```python
from build123d import *

# Parameters (mm, degrees)
SKETCH_1_W                   = 30
SKETCH_1_H                   = 40
EXTRUDE_1_DEPTH              = 9
SKETCH_2_W                   = 30
SKETCH_2_H                   = 12
EXTRUDE_2_DEPTH              = 10
HOLE_WIZARD_M4_1_D           = 4.5
HOLE_WIZARD_M4_1_CBORE_D     = 8
HOLE_WIZARD_M4_1_CBORE_DEPTH = 4.4
CHAMFER_1_SIZE               = 1
CUT_EXTRUDE_1_DEPTH          = 32.400636936


with BuildPart() as part:
    # 草图1 → 凸台-拉伸1 (new body)
    with BuildSketch(Plane(origin=(0, 0, 0), x_dir=(1, 0, 0), z_dir=(0, 1, 0))):
        Rectangle(SKETCH_1_W, SKETCH_1_H)
    extrude(amount=EXTRUDE_1_DEPTH)

    # 草图2 → 凸台-拉伸2 (add)
    with BuildSketch(Plane(origin=(0, 9, 0), x_dir=(1, 0, 0), z_dir=(0, 1, 0))):
        with Locations((0, 14)):
            Rectangle(SKETCH_2_W, SKETCH_2_H)
    extrude(amount=EXTRUDE_2_DEPTH)

    # M4 六角凹头螺钉的柱形沉头孔1 (through all)
    with Locations(Plane(origin=(0, 0, 0), x_dir=(-1, 0, 0), z_dir=(0, -1, 0))):
        with Locations((-10, 15), (10, 15)):
            CounterBoreHole(HOLE_WIZARD_M4_1_D / 2, HOLE_WIZARD_M4_1_CBORE_D / 2, HOLE_WIZARD_M4_1_CBORE_DEPTH)

    # 倒角1
    chamfer_1_edges = [part.edges().sort_by_distance(p)[0] for p in [
        (-15, 14, -8),
        (15, 14, -8),
        (-15, 9.5, -20),
        (15, 9.5, -20),
        (15, 4.5, 20),
        (-15, 4.5, 20),
    ]]
    chamfer(chamfer_1_edges, length=CHAMFER_1_SIZE)

    # 草图5 → 切除-拉伸1 (cut, through all)
    with BuildSketch(Plane.XZ):
        with BuildLine():
            Line((2.5, 20), (2.5, 10))
            ThreePointArc((2.5, 10), (0, 7.5), (-2.5, 10))
            Line((-2.5, 10), (-2.5, 20))
            ThreePointArc((-2.5, 20), (0, 22.5), (2.5, 20))
        make_face()
    extrude(amount=-CUT_EXTRUDE_1_DEPTH, mode=Mode.SUBTRACT)


solid = part.part
```
Geometry check sheet. Reference: the model listing, model coordinates, mm. A direction names the side the tool comes from. Round coordinates to 2 decimals unless told otherwise and drop trailing zeros. Loops run counter-clockwise (first coordinate to the right, second up) from the corner with the lowest first, then second, coordinate; pieces in that order, holes last. Notation, with made-up numbers: (52, 31.25) - (72, 31.25) arc R25 cw to (72, 46.25) - close; hole circle Ø10 at (77.25, 20). An arc over 180 degrees is marked (long way). Write item = value, one per line. Start each with the question number.
1. Depth check by flat-ended pin: pin 1 (8.5 mm diameter, centred on x = 1, z = 6.5, fed in from +Y); pin 2 (9 mm diameter, centred on x = 10, z = -15, fed in from -Y); pin 3 (3.5 mm diameter, centred on x = -10, z = -15, fed in from +Y); pin 4 (5 mm diameter, centred on x = 5, y = 14.5, fed in from +Z). Enter the tip coordinate at first touch or a pass-through.
2. Section check C-C on z = 14. Enter the section's corners in (x, y).
3. Thickness scan on line 1 (X direction, y = 9.75, z = -15); line 2 (X direction, y = 1, z = 11); line 3 (Z direction, x = 10, y = 12.5). Record the ranges inside material, lowest first.
4. Section check A-A on y = 11. Enter the section's corners in (x, z).
5. Section check D-D on x = -4.5. Enter the section's corners in (y, z), then the cut area to 3 significant figures.
6. Section check B-B on x = -10. Enter the section's corners in (y, z).
7. Set-up check for faces 4 (the face through (-14.5, 13.9, -8.5)), 5 (the face through (0, 0, 0)), 6 (the face through (0, 14, -8)), 7 (the face through (-2.5, 4, 15)), 8 (the face through (8, 4.4, -13)): record each of +Z, -Z, +X, -X, +Y, -Y from which the full face is reachable in a straight line by a thin tool's end or side.
8. Mould release check, pull along X, two halves, no side actions. Record for faces 1 (the face through (-14.5, 9.6, -19.5)), 2 (the face through (10.521, 2.169, -18.966)), 3 (the face through (14.5, 13.9, -8.5)): released by +X, released by -X, zero draft, split by the parting line, or undercut.
Working result:
q1.pin_1 = 9
q1.pin_2 = 0
q1.pin_3 = through
q1.pin_4 = -8
q2.outline = (-15, 0) - (-2.5, 0) - (-2.5, 9) - (-15, 9) - close; (2.5, 0) - (15, 0) - (15, 9) - (2.5, 9) - close
q3.line_1 = -15 to -12.25, -7.75 to 7.75, 12.25 to 15
q3.line_2 = -15 to -2.5, 2.5 to 15
q3.line_3 = -20 to -17.25, -12.75 to -8
q4.outline = (-15, -19) - (-14, -20) - (14, -20) - (15, -19) - (15, -9) - (14, -8) - (-14, -8) - (-15, -9) - close; hole circle Ø4.5 at (-10, -15); hole circle Ø4.5 at (10, -15)
q5.outline = (0, -20) - (19, -20) - (19, -8) - (9, -8) - (9, 20) - (0, 20) - close
q5.area = 480 mm^2
q6.outline = (0, -20) - (19, -20) - (19, -17.25) - (4.4, -17.25) - (4.4, -19) - (0, -19) - close; (0, -11) - (4.4, -11) - (4.4, -12.75) - (19, -12.75) - (19, -8) - (9, -8) - (9, 20) - (0, 20) - close
q7.face_4 = +Z, -X, +Y
q7.face_5 = +Z, -Z, +X, -X, -Y
q7.face_6 = +Z, +X, -X, +Y
q7.face_7 = +Z, +Y, -Y
q7.face_8 = -Y
q8.face_1 = released by -X
q8.face_2 = undercut
q8.face_3 = released by +X
